Can you work these out from the model? Positions are in its coordinate system, mm. A direction names the side the tool comes from. Give positions to 0.01 mm unless a question says otherwise; leave off trailing zeros. Write each loop counter-clockwise with the first axis right and the second up, starting at its lowest first coordinate (ties: lowest second). Pieces come first, ordered by that corner, then holes.
```python
from build123d import *

# Parameters (mm, degrees)
SKETCH_1_R          = 32
EXTRUDE_1_DEPTH     = 14
EXTRUDE_2_DEPTH     = 11
SKETCH_3_R          = 5
CUT_EXTRUDE_1_DEPTH = 59.959732021
SKETCH_4_R          = 7.5
CUT_EXTRUDE_2_DEPTH = 3
SKETCH_5_R          = 17.5
EXTRUDE_3_DEPTH     = 24.5
SKETCH_6_R          = 20
CUT_EXTRUDE_3_DEPTH = 7
EXTRUDE_START       = 3.5
SKETCH_7_R          = 17.5
EXTRUDE_4_DEPTH     = 3.5
SKETCH_8_R          = 12.5
CUT_EXTRUDE_4_DEPTH = 63.293659388


with BuildPart() as part:
    # 草图1 → 凸台-拉伸1 (new body)
    with BuildSketch(Plane(origin=(0, 0, 0), x_dir=(1, 0, 0), z_dir=(0, 1, 0))):
        with Locations(Location((0, 0, 0), (0, 0, 270))):
            Circle(SKETCH_1_R)
    extrude(amount=EXTRUDE_1_DEPTH)

    # 草图2 → 凸台-拉伸2 (add)
    with BuildSketch(Plane(origin=(0, 0, 0), x_dir=(1, 0, 0), z_dir=(0, 1, 0))):
        with BuildLine():
            Line((42.928542082, 8.398269516), (24.979991994, 20))
            ThreePointArc((24.979991994, 20), (32, 0), (24.979991994, -20))
            Line((24.979991994, -20), (42.928542082, -8.398269516))
            ThreePointArc((42.928542082, -8.398269516), (47.5, 0), (42.928542082, 8.398269516))
        make_face()
    extrude_2 = extrude(amount=EXTRUDE_2_DEPTH)

    # 镜向1: 凸台-拉伸2 across plane
    add(extrude_2.mirror(Plane(origin=(0, 0, 0), x_dir=(0, 0, 1), z_dir=(1, 0, 0))))

    # 草图3 → 切除-拉伸1 (cut, through all)
    with BuildSketch(Plane(origin=(0, 0, 0), x_dir=(1, 0, 0), z_dir=(0, 1, 0))):
        with Locations(Location((-38, 0, 0), (0, 0, 270))):
            Circle(SKETCH_3_R)
        with Locations(Location((38, 0, 0), (0, 0, 270))):
            Circle(SKETCH_3_R)
    extrude(amount=CUT_EXTRUDE_1_DEPTH, mode=Mode.SUBTRACT)

    # 草图4 → 切除-拉伸2 (cut)
    with BuildSketch(Plane(origin=(0, 14, 0), x_dir=(1, 0, 0), z_dir=(0, 1, 0))):
        with Locations((-38, 0)):
            Circle(SKETCH_4_R)
        with Locations((38, 0)):
            Circle(SKETCH_4_R)
    extrude(amount=-CUT_EXTRUDE_2_DEPTH, mode=Mode.SUBTRACT)

    # 草图5 → 凸台-拉伸3 (add)
    with BuildSketch(Plane(origin=(0, 0, 0), x_dir=(1, 0, 0), z_dir=(0, 1, 0))):
        with Locations(Location((0, 0, 0), (0, 0, 270))):
            Circle(SKETCH_5_R)
    extrude(amount=EXTRUDE_3_DEPTH)

    # 草图6 → 切除-拉伸3 (cut)
    with BuildSketch(Plane.XZ):
        with Locations(Location((0, 0, 0), (0, 0, 270))):
            Circle(SKETCH_6_R)
    extrude(amount=-CUT_EXTRUDE_3_DEPTH, mode=Mode.SUBTRACT)

    # 草图7 → 凸台-拉伸4 (add)
    with BuildSketch(Plane.XZ.offset(-7).offset(EXTRUDE_START)):
        with Locations(Location((0, 0, 0), (0, 0, 90))):
            Circle(SKETCH_7_R)
    extrude(amount=-EXTRUDE_4_DEPTH)

    # 草图8 → 切除-拉伸4 (cut, through all)
    with BuildSketch(Plane(origin=(0, 24.5, 0), x_dir=(1, 0, 0), z_dir=(0, 1, 0))):
        with Locations(Location((0, 0, 0), (0, 0, 270))):
            Circle(SKETCH_8_R)
    extrude(amount=-CUT_EXTRUDE_4_DEPTH, mode=Mode.SUBTRACT)


solid = part.part
```
1) Suppose I cut it at D-D on y = 22. Write out the boundary of the cut face in (x, z), plus the area to 3 significant figures.
Values follow:
outline: circle Ø35 at (0, 0); hole circle Ø25 at (0, 0)
area: 471 mm2
2) Suppose I cut it at A-A on x = 0. Write out the boundary of the cut face in (y, z), plus the area to 3 significant figures.
Values follow:
outline: (0, -32) - (14, -32) - (14, -17.5) - (24.5, -17.5) - (24.5, -12.5) - (3.5, -12.5) - (3.5, -17.5) - (7, -17.5) - (7, -20) - (0, -20) - close; (0, 20) - (7, 20) - (7, 17.5) - (3.5, 17.5) - (3.5, 12.5) - (24.5, 12.5) - (24.5, 17.5) - (14, 17.5) - (14, 32) - (0, 32) - close
area: 581 mm2
3) For faces 4 (the face through (0.646, 8.458, -31.993)), 5 (the face through (-0.646, 8.458, 31.993)), 6 (the face through (-30.5, 12.5, 0.1)), 7 (the face through (-19.524, 3.451, 4.336)), which set-ups out of +Z, -Z, +X, -X, +Y, -Y let a thin tool reach every point of the face, with its end or its side?
Values follow:
face 4: -Z, +Y
face 5: +Z, +Y
face 6: -X, +Y
face 7: -Y
4) If we mould it in two halves opening along X, with no side actions, what happens to faces 1 (the face through (10.648, 5.226, -13.887)), 2 (the face through (-33.8, 5.4, 14.3)), 3 (the face through (32.9, 11, 1.4))? For each: +X half, -X half, draft (parallel to the pull), parting line (faces both ways), or undercut.
Values follow:
face 1: undercut
face 2: -X half
face 3: draft
5) Suppose I cut it at C-C on z = 0. State how many separate pieces and enclosed holes the cut face has, plus the area to 3 significant figures.
Values follow:
separate pieces: 4
enclosed holes: 0
area: 693 mm2
6) Suppose I cut it at B-B on y = 2.5. Write out the boundary of the cut face in (x, z), plus the area to 3 significant figures.
Values follow:
outline: (-42.93, -8.4) - (-24.98, -20) arc R32 ccw to (24.98, -20) - (42.93, -8.4) arc R10 ccw to (42.93, 8.4) - (24.98, 20) arc R32 ccw to (-24.98, 20) - (-42.93, 8.4) arc R10 ccw to start; hole circle Ø10 at (-38, 0); hole circle Ø40 at (0, 0); hole circle Ø10 at (38, 0)
area: 2,550 mm2
7) For pin 1 Ø7 at (x, z) = (-41, 1) entering from +Y; pin 2 Ø6 at (x, z) = (38, 0) entering from +Y; pin 3 Ø18 at (x, z) = (31, -9) entering from +Y; pin 4 Ø8 at (x, y) = (8.5, 21.5) entering from -Z, each with a flat end and sliding along its axis, tell me the tip position at first contact or that it passes through.
Values follow:
pin 1: stops at y = 11
pin 2: passes through
pin 3: stops at y = 14
pin 4: stops at z = -16.91
8) Please list where these lines run through material, in increasing order: L1, parallel to X at y = 8.25, z = 0; L2, parallel to X at y = 5.25, z = 0; L3, parallel to X at y = 12.75, z = 0.
Values follow:
L1: x = -47.5 to -43, -33 to -12.5, 12.5 to 33, 43 to 47.5
L2: x = -47.5 to -43, -33 to -20, -17.5 to -12.5, 12.5 to 17.5, 20 to 33, 43 to 47.5
L3: x = -30.5 to -12.5, 12.5 to 30.5
